Verification items for the finished model (mm, model axes). A direction names the side the tool comes from. Give positions to 0.01 mm unless a question says otherwise; leave off trailing zeros. Write each loop counter-clockwise with the first axis right and the second up, starting at its lowest first coordinate (ties: lowest second). Pieces come first, ordered by that corner, then holes. Notation, with made-up numbers: M 82,65.5 L 139,65.5 A16 cw 139,91.5 Z; hole C 61.25,88.5 d9. An arc over 180 degrees is marked long. Answer as a JSON object with one key per item and string values.
```python
from build123d import *

# Parameters (mm, degrees)
SKETCH_1_W           = 100
SKETCH_1_H           = 120
BOSS_EXTRUDE_1_DEPTH = 30
SKETCH_2_R           = 27.5
BOSS_EXTRUDE_2_DEPTH = 30
SKETCH_4_W           = 15
SKETCH_4_H           = 30
BOSS_EXTRUDE_3_DEPTH = 30
SKETCH_5_W           = 100
SKETCH_5_H           = 300
SKETCH_5_R           = 15
BOSS_EXTRUDE_4_DEPTH = 30
FILLET_1_R           = 30


with BuildPart() as part:
    # Sketch 1 → Boss-Extrude 1 (new body)
    with BuildSketch(Plane(origin=(0, 0, 0), x_dir=(1, 0, 0), z_dir=(0, 1, 0))):
        Rectangle(SKETCH_1_W, SKETCH_1_H)
    extrude(amount=BOSS_EXTRUDE_1_DEPTH)

    # Sketch 2 → Boss-Extrude 2 (add)
    with BuildSketch(Plane.XY.offset(60)):
        with BuildLine():
            Line((-44.961585181, 151.858993825), (-50, 30))
            Line((-50, 30), (50, 30))
            Line((50, 30), (44.961585181, 151.858993825))
            ThreePointArc((44.961585181, 151.858993825), (0, 195), (-44.961585181, 151.858993825))
        make_face()
        with Locations((0, 150)):
            Circle(SKETCH_2_R, mode=Mode.SUBTRACT)
    boss_extrude_2 = extrude(amount=-BOSS_EXTRUDE_2_DEPTH)

    # Sketch 4 → Boss-Extrude 3 (add)
    with BuildSketch(Plane.XY.offset(60)):
        with Locations((0, 15)):
            Rectangle(SKETCH_4_W, SKETCH_4_H)
    boss_extrude_3 = extrude(amount=BOSS_EXTRUDE_3_DEPTH)

    # Mirror 1: Boss-Extrude 2, Boss-Extrude 3 across plane
    add(boss_extrude_2.mirror(Plane.XY))
    add(boss_extrude_3.mirror(Plane.XY))

    # Sketch 5 → Boss-Extrude 4 (add)
    with BuildSketch(Plane.XZ):
        Rectangle(SKETCH_5_W, SKETCH_5_H)
        with Locations(Location((0, -105, 0), (0, 0, 270))):
            Circle(SKETCH_5_R, mode=Mode.SUBTRACT)
        with Locations(Location((0, 105, 0), (0, 0, 270))):
            Circle(SKETCH_5_R, mode=Mode.SUBTRACT)
    extrude(amount=-BOSS_EXTRUDE_4_DEPTH)

    # Fillet 1
    fillet_1_edges = [part.edges().sort_by_distance(p)[0] for p in [
        (-50, 15, -150),
        (50, 15, 150),
        (50, 15, -150),
        (-50, 15, 150),
    ]]
    fillet(fillet_1_edges, radius=FILLET_1_R)


solid = part.part
```
1) Access from +Z, -Z, +X, -X, +Y, -Y to the whole of each face (thin tool, end or side, straight path). Record for faces 1 (the face through (-12, 30, 116)), 2 (the face through (0, 15, -150)), 3 (the face through (-1, 95, -60)), 4 (the face through (-1, 95, 30)).
Completed:
{"face 1": "+Z, +X, -X, +Y", "face 2": "-Z, +X, -X, +Y, -Y", "face 3": "-Z, +X, -X, +Y", "face 4": "+X, -X, +Y"}
2) Section check B-B on z = -105. Record the boundary of the cut face in (x, y).
Completed:
{"outline": "M -50,0 L -15,0 L -15,30 L -50,30 Z; M 15,0 L 50,0 L 50,30 L 15,30 Z"}
3) Section check D-D on z = -47.5. Record the boundary of the cut face in (x, y), and give its area (3 significant figures).
Completed:
{"outline": "M -50,0 L 50,0 L 50,30 L 44.96,151.86 A45 ccw -44.96,151.86 L -50,30 Z; hole C 0,150 d55", "area": "15,200 mm2"}
4) Thickness scan on L1, parallel to Z at x = -26.5, y = 110; L2, parallel to Y at x = -22, z = -79; L3, parallel to X at y = 20.75, z = 105. Record the ranges inside material, lowest first.
Completed:
{"L1": "z = -60 to -30, 30 to 60", "L2": "y = 0 to 30", "L3": "x = -50 to -15, 15 to 50"}
5) Section check C-C on y = 45. Record the boundary of the cut face in (x, z).
Completed:
{"outline": "M -49.38,-60 L 49.38,-60 L 49.38,-30 L -49.38,-30 Z; M -49.38,30 L 49.38,30 L 49.38,60 L -49.38,60 Z"}
6) Go/stop test with flat-tipped pins: pin 1 (18 mm diameter, centred on x = 5, z = -12.5, fed in from +Y); pin 2 (1 mm diameter, centred on y = 109.5, z = 36, fed in from +X); pin 3 (4 mm diameter, centred on y = 174, z = 33.5, fed in from +X). Record where each tip stops, or that it passes through.
Completed:
{"pin 1": "stops at y = 30", "pin 2": "stops at x = 46.73", "pin 3": "stops at x = 39.26"}
7) Release check for a two-part mould opening along X. For faces 5 (the face through (-3.58, 177.266, 45.21)), 6 (the face through (12.65, 14.79, -113.06)), 7 (the face through (40.979, 15.21, 141.445)), 8 (the face through (0, 15, 150)) record: pulls with the +X half, pulls with the -X half, needs draft (parallel to the pull), parting line crosses it, or undercut.
Completed:
{"face 5": "undercut", "face 6": "undercut", "face 7": "pulls with the +X half", "face 8": "needs draft"}
8) Section check A-A on x = 0. Record the boundary of the cut face in (y, z).
Completed:
{"outline": "M 0,-150 L 30,-150 L 30,-120 L 0,-120 Z; M 0,-90 L 30,-90 L 30,-60 L 122.5,-60 L 122.5,-30 L 30,-30 L 30,30 L 122.5,30 L 122.5,60 L 30,60 L 30,90 L 0,90 Z; M 0,120 L 30,120 L 30,150 L 0,150 Z; M 177.5,-60 L 195,-60 L 195,-30 L 177.5,-30 Z; M 177.5,30 L 195,30 L 195,60 L 177.5,60 Z"}
